Here's how the part is built. I have some questions about the finished solid (model axes, mm). A direction names the side the tool comes from. Coordinates: 2 decimals unless noted, no trailing zeros. Write each loop counter-clockwise with the first axis right and the second up, starting at its lowest first coordinate (ties: lowest second). Pieces come first, ordered by that corner, then holes.
Item 1: If we mould it in two halves opening along Y, with no side actions, what happens to faces 1 (the face through (0, -26, 550)), 2 (the face through (0, 30, 550)), 3 (the face through (30, 0, 550)), 4 (the face through (0, 26, 550))? For each: pulls with the +Y half, pulls with the -Y half, needs draft (parallel to the pull), parting line crosses it, or undercut.
Item 2: I want a section at A-A (x = -5). Please give me the cut outline in (y, z).
Item 3: Please list where these lines run through material, in increasing order: line 1 (X direction, y = -15, z = 786.5); line 2 (Y direction, x = 27, z = 839.5).
Item 4: I want a section at C-C (z = 743). Please give me the cut outline in (x, y).
Item 5: For faces 5 (the face through (-27, 0, 0)), 6 (the face through (26, 0, 550)), which set-ups out of +Z, -Z, +X, -X, +Y, -Y let a thin tool reach every point of the face, with its end or its side?
from build123d import *

# Parameters (mm, degrees)
SKETCH1_W           = 60
SKETCH1_H           = 60
BOSS_EXTRUDE1_DEPTH = 1116
FILLET1_R           = 5
SHELL1_T            = -4


with BuildPart() as part:
    # Sketch1 → Boss-Extrude1 (new body)
    with BuildSketch(Plane.XY):
        Rectangle(SKETCH1_W, SKETCH1_H)
    extrude(amount=BOSS_EXTRUDE1_DEPTH)

    # Fillet1
    fillet1_edges = [part.edges().sort_by_distance(p)[0] for p in [
        (30, -30, 558),
        (30, 30, 558),
        (-30, 30, 558),
        (-30, -30, 558),
    ]]
    fillet(fillet1_edges, radius=FILLET1_R)

    # Shell1
    shell1_openings = [part.faces().sort_by_distance(p)[0] for p in [
        (0, 0, 1116),
        (0, 0, 0),
    ]]
    offset(amount=SHELL1_T, openings=shell1_openings, kind=Kind.INTERSECTION)


solid = part.part
Answer:
1. face 1: undercut
1. face 2: pulls with the +Y half
1. face 3: needs draft
1. face 4: undercut
2. outline: (-30, 0) - (-26, 0) - (-26, 1116) - (-30, 1116) - close; (26, 0) - (30, 0) - (30, 1116) - (26, 1116) - close
3. line 1: x = -30 to -26, 26 to 30
3. line 2: y = -29.58 to 29.58
4. outline: (-30, -25) arc R5 ccw to (-25, -30) - (25, -30) arc R5 ccw to (30, -25) - (30, 25) arc R5 ccw to (25, 30) - (-25, 30) arc R5 ccw to (-30, 25) - close; hole (-26, -25) arc R1 ccw to (-25, -26) - (25, -26) arc R1 ccw to (26, -25) - (26, 25) arc R1 ccw to (25, 26) - (-25, 26) arc R1 ccw to (-26, 25) - close
5. face 5: -Z, +X, -X, +Y, -Y
5. face 6: +Z, -Z
